from build123d import *

# Parameters (mm, degrees)
SKETCH_1_W          = 880
SKETCH_1_H          = 2266
EXTRUDE_1_DEPTH     = 40
SKETCH_2_W          = 300
SKETCH_2_H          = 340.469439268
CUT_EXTRUDE_1_DEPTH = 1217.095802147
SKETCH_3_W          = 300
SKETCH_3_H          = 426.530560732
CUT_EXTRUDE_2_DEPTH = 1217.095802147
SKETCH_4_W          = 300
SKETCH_4_H          = 340.469439268
CUT_EXTRUDE_3_DEPTH = 1217.095802147
SKETCH_5_W          = 580
SKETCH_5_H          = 404.015280366
CUT_EXTRUDE_4_DEPTH = 1217.095802147
FILLET_2_R          = 100
FILLET_3_R          = 30


with BuildPart() as part:
    # 草图1 → 凸台-拉伸1 (new body)
    with BuildSketch(Plane(origin=(0, 0, 0), x_dir=(1, 0, 0), z_dir=(0, 1, 0))):
        Rectangle(SKETCH_1_W, SKETCH_1_H)
    extrude(amount=EXTRUDE_1_DEPTH)

    # 草图2 → 切除-拉伸1 (cut, through all)
    with BuildSketch(Plane.XZ):
        with Locations((0, 208.75)):
            Rectangle(SKETCH_2_W, SKETCH_2_H)
    extrude(amount=-CUT_EXTRUDE_1_DEPTH, mode=Mode.SUBTRACT)

    # 草图3 → 切除-拉伸2 (cut, through all)
    with BuildSketch(Plane.XZ):
        with Locations((0, -352.75)):
            Rectangle(SKETCH_3_W, SKETCH_3_H)
    extrude(amount=-CUT_EXTRUDE_2_DEPTH, mode=Mode.SUBTRACT)

    # 草图4 → 切除-拉伸3 (cut, through all)
    with BuildSketch(Plane(origin=(0, 0, 0), x_dir=(-1, 0, 0), z_dir=(0, -1, 0))):
        with Locations((0, 914.25)):
            Rectangle(SKETCH_4_W, SKETCH_4_H)
    extrude(amount=-CUT_EXTRUDE_3_DEPTH, mode=Mode.SUBTRACT)

    # 草图5 → 切除-拉伸4 (cut, through all)
    with BuildSketch(Plane.XZ):
        with Locations((0, 780.992359817)):
            Rectangle(SKETCH_5_W, SKETCH_5_H)
    extrude(amount=-CUT_EXTRUDE_4_DEPTH, mode=Mode.SUBTRACT)

    # 圆角2
    fillet_2_edges = [part.edges().sort_by_distance(p)[0] for p in [
        (-290, 20, 578.984719634),
        (-290, 20, 983),
        (290, 20, 983),
        (290, 20, 578.984719634),
    ]]
    fillet(fillet_2_edges, radius=FILLET_2_R)

    # 圆角3
    fillet_3_edges = [part.edges().sort_by_distance(p)[0] for p in [
        (-150, 20, 38.515280366),
        (-150, 20, 378.984719634),
        (150, 20, 378.984719634),
        (150, 20, 38.515280366),
        (-150, 20, -566.015280366),
        (-150, 20, -139.484719634),
        (150, 20, -139.484719634),
        (150, 20, -566.015280366),
        (-150, 20, -1084.484719634),
        (-150, 20, -744.015280366),
        (150, 20, -744.015280366),
        (150, 20, -1084.484719634),
    ]]
    fillet(fillet_3_edges, radius=FILLET_3_R)


solid = part.part
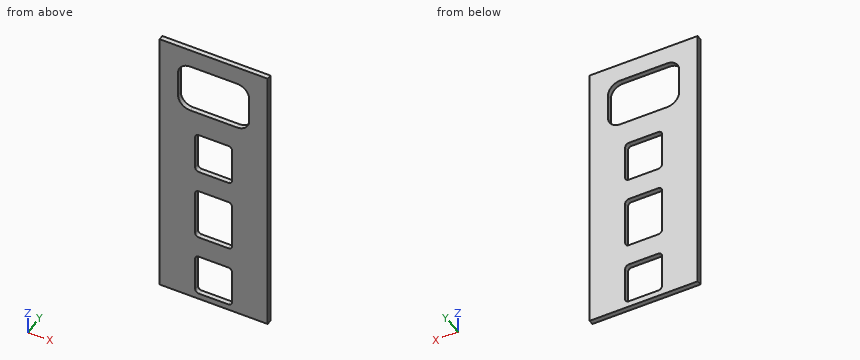
The listing builds one solid part. Answer for the finished solid, in the listing's coordinates (mm). Give positions to 0.01 mm unless a question says otherwise; leave off trailing zeros. Order: outer loops, then holes, each group sorted by start corner. A loop starts at its lowest first (then second) coordinate and runs counter-clockwise, first axis right, second up. Notation, with made-up numbers: (-14.75, -18.75) - (28.25, -18.75) arc R27 ccw to (28.25, 14.25) - close; hole circle Ø1 at (55.5, 0). An arc over 180 degrees is marked (long way). Use one line per item in the form item = value.
1) Find section B-B on z = -216.5. Determine the outline of the cut face in (x, y), and give its area (3 significant figures).
Verdict:
outline = (-440, 0) - (-150, 0) - (-150, 40) - (-440, 40) - close; (150, 0) - (440, 0) - (440, 40) - (150, 40) - close
area = 23,200 mm^2
2) Find section C-C on y = 20. Give the number of separate pieces and of enclosed holes in the cut face, and give its area (3 significant figures).
Verdict:
separate_pieces = 1
enclosed_holes = 4
area = 1,440,000 mm^2
3) This flat-tipped pin is pushed along its axis until it touches: pin 1 (5 mm diameter, centred on x = 311.5, z = -513.5, fed in from -Y). Where does it stop, or does it pass through?
Verdict:
pin_1 = 0
4) Consider probe 1 along Z at (x, y) = (-95.5, 18.5); probe 2 along X at (y, z) = (3, 771); probe 3 along X at (y, z) = (37.5, -437). Determine where each line is inside the solid, lowest interval first. Write a range as [from, to].
Verdict:
probe_1 = [-1133, -1084.48], [-744.02, -566.02], [-139.48, 38.52], [378.98, 578.98], [983, 1133]
probe_2 = [-440, -290], [290, 440]
probe_3 = [-440, -150], [150, 440]
5) Find section D-D on z = 655. Determine the outline of the cut face in (x, y), and give its area (3 significant figures).
Verdict:
outline = (-440, 0) - (-287.08, 0) - (-287.08, 40) - (-440, 40) - close; (287.08, 0) - (440, 0) - (440, 40) - (287.08, 40) - close
area = 12,200 mm^2
6) Find section A-A on x = 82. Determine the outline of the cut face in (y, z).
Verdict:
outline = (0, -1133) - (40, -1133) - (40, -1084.48) - (0, -1084.48) - close; (0, -744.02) - (40, -744.02) - (40, -566.02) - (0, -566.02) - close; (0, -139.48) - (40, -139.48) - (40, 38.52) - (0, 38.52) - close; (0, 378.98) - (40, 378.98) - (40, 578.98) - (0, 578.98) - close; (0, 983) - (40, 983) - (40, 1133) - (0, 1133) - close
